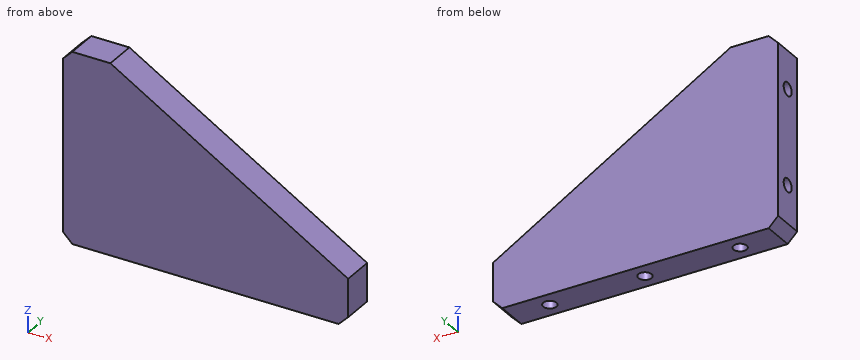
from build123d import *

# Parameters (mm, degrees)
SKETCH_1_W             = 90
SKETCH_1_H             = 60
EXTRUDE_1_DEPTH        = 10
CUT_EXTRUDE_1_DEPTH    = 15
CHAMFER_1_SIZE         = 3
HOLE_WIZARD_M5_1_D     = 4.2
HOLE_WIZARD_M5_1_DEPTH = 12.4
HOLE_WIZARD_M5_1_TIP   = 1.2618073
HOLE_WIZARD_M5_2_D     = 4.2
HOLE_WIZARD_M5_2_DEPTH = 12.4
HOLE_WIZARD_M5_2_TIP   = 1.2618073


with BuildPart() as part:
    # 草图1 → 凸台-拉伸1 (new body)
    with BuildSketch(Plane(origin=(0, 0, 0), x_dir=(1, 0, 0), z_dir=(0, 1, 0))):
        Rectangle(SKETCH_1_W, SKETCH_1_H)
    extrude(amount=EXTRUDE_1_DEPTH)

    # 草图2 → 切除-拉伸1 (cut)
    with BuildSketch(Plane(origin=(0, 10, 0), x_dir=(1, 0, 0), z_dir=(0, 1, 0))):
        Polygon((45, 15), (-30, -30), (45, -30), align=None)
    extrude(amount=-CUT_EXTRUDE_1_DEPTH, mode=Mode.SUBTRACT)

    # 倒角1
    chamfer_1_edges = [part.edges().sort_by_distance(p)[0] for p in [
        (-45, 5, 30),
        (-45, 5, -30),
        (45, 5, -30),
    ]]
    chamfer(chamfer_1_edges, length=CHAMFER_1_SIZE)

    # M5 螺纹孔1
    with Locations(Plane.ZY.offset(45)):
        with Locations((-15, 5), (15, 5)):
            Hole(HOLE_WIZARD_M5_1_D / 2, depth=HOLE_WIZARD_M5_1_DEPTH)
            with Locations((0, 0, -(HOLE_WIZARD_M5_1_DEPTH + HOLE_WIZARD_M5_1_TIP / 2))):  # 118° drill point
                Cone(0, HOLE_WIZARD_M5_1_D / 2, HOLE_WIZARD_M5_1_TIP, mode=Mode.SUBTRACT)

    # M5 螺纹孔2
    with Locations(Plane(origin=(0, 0, -30), x_dir=(-1, 0, 0), z_dir=(0, 0, -1))):
        with Locations((30, 5), (0, 5), (-30, 5)):
            Hole(HOLE_WIZARD_M5_2_D / 2, depth=HOLE_WIZARD_M5_2_DEPTH)
            with Locations((0, 0, -(HOLE_WIZARD_M5_2_DEPTH + HOLE_WIZARD_M5_2_TIP / 2))):  # 118° drill point
                Cone(0, HOLE_WIZARD_M5_2_D / 2, HOLE_WIZARD_M5_2_TIP, mode=Mode.SUBTRACT)


solid = part.part
Design review of the part built by this model. Coordinates are the model's own, in mm. Round coordinates to 2 decimals unless told otherwise and drop trailing zeros. Loops run counter-clockwise (first coordinate to the right, second up) from the corner with the lowest first, then second, coordinate; pieces in that order, holes last. Notation, with made-up numbers: M 7,-27.75 L 11,-27.75 A25 cw 11,1.25 Z; hole C 69,67.5 d2. An arc over 180 degrees is marked long. Answer as a JSON object with one key per item and string values.
Item 1: Wall thickness on L1, parallel to X at y = 5, z = -25.25; L2, parallel to Z at x = -33, y = 6.5; L3, parallel to Y at x = 30, z = -24: over which ranges is each line inside the solid? List them lowest first. Write a range as from..to.
Answer sheet:
{"L1": "x = -45..-32.1, -27.9..-2.1, 2.1..27.9, 32.1..45", "L2": "z = -30..-16.47, -13.53..13.53, 16.47..30", "L3": "y = 0..2.9, 7.1..10"}
Item 2: Clearance check with flat-ended pins moving along their axes: P1, Ø1, axis at y = 2, z = -2, coming from the +X side; P2, Ø2.5, axis at y = 5, z = -15, coming from the -X side; P3, Ø5.5, axis at y = 5, z = 15, coming from the +X side. State where each tip first meets the part, or that it passes through.
Answer sheet:
{"P1": "stops at x = 24.17", "P2": "stops at x = -32.09", "P3": "stops at x = -0.42"}
Item 3: We need section B-B on z = 19.5. Give the boundary of the cut face in (x, y), and give its area (3 significant figures).
Answer sheet:
{"outline": "M -45,0 L -12.5,0 L -12.5,10 L -45,10 Z", "area": "325 mm^2"}
Item 4: We need section A-A on x = -25.5. Give the boundary of the cut face in (y, z).
Answer sheet:
{"outline": "M 0,-30 L 10,-30 L 10,27.3 L 0,27.3 Z"}
